Verification items for this drawing (mm, ordinates from the low corner). Round coordinates to 2 decimals unless told otherwise and drop trailing zeros. Order: outer loops, then holes, each group sorted by start corner. A loop starts at its lowest first (then second) coordinate and runs counter-clockwise, first axis right, second up. Notation, with made-up numbers: M -24,2.5 L 30,2.5 A33 cw 30,31.5 Z; hole C 61.25,61 d11. An arc over 180 degrees is marked long. Return JSON: item names as keys, results as strings. Group by question number.
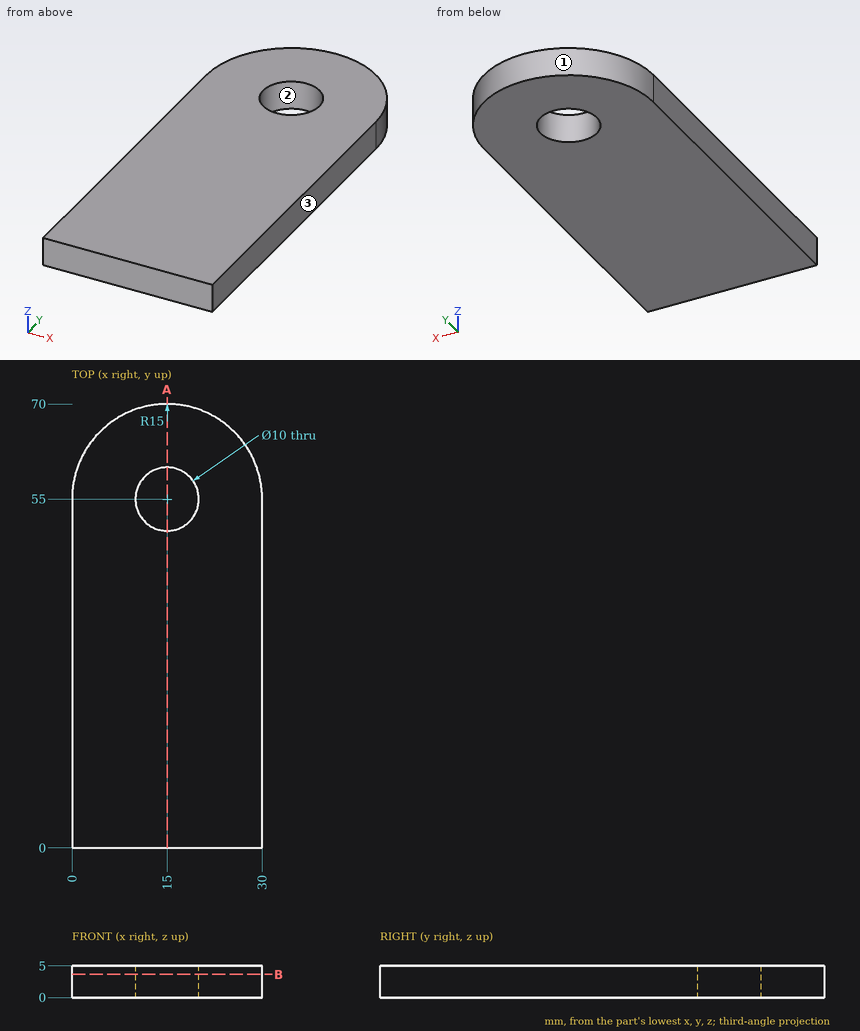
1. Draft check along X on the marked faces 1, 2 and 3. Enter one of: +X half, -X half, draft (parallel to the pull), parting line (faces both ways), or undercut.
2. Cross-section at A-A (x = 15). Enter the section's corners in (y, z).
3. Go/stop test with flat-tipped pins: pin 1 (1.5 mm diameter, centred on x = 7.5, z = 3, fed in from +Y); pin 2 (2 mm diameter, centred on x = 16.5, z = 3.5, fed in from +Y). Record where each tip stops, or that it passes through.
4. Cross-section at B-B (z = 3.65). Enter the section's corners in (x, y).
5. Thickness scan on line 1 along Y through (x, z) = (15, 2.35); line 2 along Y through (x, z) = (16.75, 1.9); line 3 along Y through (x, z) = (7.25, 0.45). Record the ranges inside material, lowest first. Write a range as from..to.
Computed:
{
 "1": {"face 1": "parting line", "face 2": "undercut", "face 3": "+X half"},
 "2": {"outline": "M 0,0 L 50,0 L 50,5 L 0,5 Z; M 60,0 L 70,0 L 70,5 L 60,5 Z"},
 "3": {"pin 1": "stops at y = 68.4", "pin 2": "stops at y = 69.99"},
 "4": {"outline": "M 0,0 L 30,0 L 30,55 A15 ccw 0,55 Z; hole C 15,55 d10"},
 "5": {"line 1": "y = 0..50, 60..70", "line 2": "y = 0..50.32, 59.68..69.9", "line 3": "y = 0..67.84"}
}
